Could you check a few things on this drawing? It's one solid part, dimensions in mm from its lowest x, y, z. Round coordinates to 2 decimals unless told otherwise and drop trailing zeros. Write each loop counter-clockwise with the first axis right and the second up, starting at its lowest first coordinate (ties: lowest second). Pieces come first, ordered by that corner, then holes. Notation, with made-up numbers: (-10.5, -28.75) -> (26.5, -28.75) arc R12 ccw to (26.5, -12.75) -> close; hole circle Ø2 at (73.25, -14.5). An arc over 180 degrees is marked (long way). Answer in a Markdown table with one row per item.
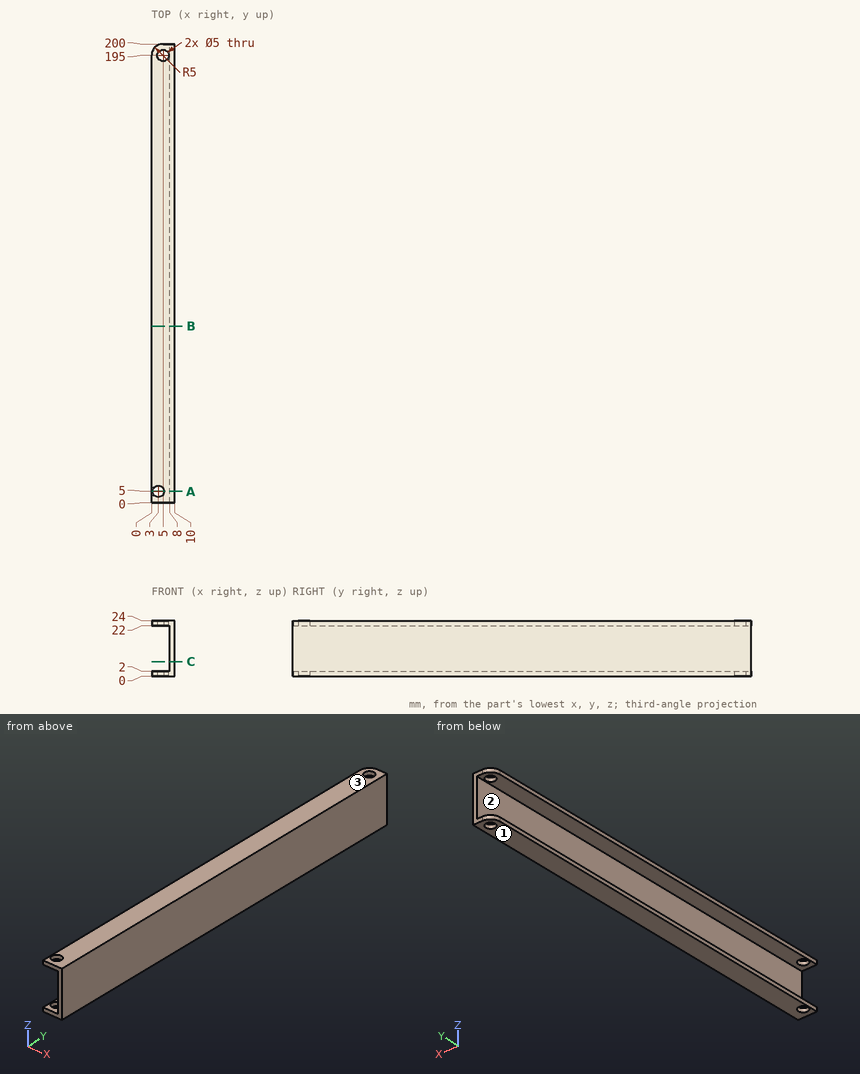
1) Thinking about a two-plate mould opening in Z: for the marked faces 1, 2 and 3, which applies, +Z half, -Z half, draft (parallel to the pull), parting line (faces both ways), or undercut?
Findings:
| item | result |
|---|---|
| face 1 | -Z half |
| face 2 | undercut |
| face 3 | +Z half |
2) Please list where these lines run through material, in increasing order: line 1 (Z direction, x = 6.75, y = 85.5); line 2 (X direction, y = 5, z = 23.1); line 3 (Y direction, x = 5, z = 1.4).
Findings:
| item | result |
|---|---|
| line 1 | z = 0 to 2, 22 to 24 |
| line 2 | x = 0 to 0.5, 5.5 to 10 |
| line 3 | y = 0 to 3.5, 6.5 to 192.5, 197.5 to 200 |
3) Imagine slicing it at B-B, the plane y = 77. Please give me the cut outline in (x, z).
Findings:
| item | result |
|---|---|
| outline | (0, 0) -> (10, 0) -> (10, 24) -> (0, 24) -> (0, 22) -> (8, 22) -> (8, 2) -> (0, 2) -> close |
4) Imagine slicing it at C-C, the plane z = 6.25. Please give me the cut outline in (x, y), plus the area to 3 significant figures.
Findings:
| item | result |
|---|---|
| outline | (8, 0) -> (10, 0) -> (10, 200) -> (8, 200) -> close |
| area | 400 mm^2 |
5) Imagine slicing it at A-A, the plane y = 5. Please give me the cut outline in (x, z), plus the area to 3 significant figures.
Findings:
| item | result |
|---|---|
| outline | (0, 0) -> (0.5, 0) -> (0.5, 2) -> (0, 2) -> close; (0, 22) -> (0.5, 22) -> (0.5, 24) -> (0, 24) -> close; (5.5, 0) -> (10, 0) -> (10, 24) -> (5.5, 24) -> (5.5, 22) -> (8, 22) -> (8, 2) -> (5.5, 2) -> close |
| area | 60.0 mm^2 |
6) For pin 1 (5 mm diameter, centred on x = 3, z = 18, fed in from -Y); pin 2 (1 mm diameter, centred on y = 102.5, z = 9, fed in from -X), each with a flat end and sliding along its axis, tell me the tip position at first contact or that it passes through.
Findings:
| item | result |
|---|---|
| pin 1 | passes through |
| pin 2 | stops at x = 8 |
